Work out the finished part from the listing and answer in its coordinate system (mm). A direction names the side the tool comes from. Coordinates: 2 decimals unless noted, no trailing zeros. Order: outer loops, then holes, each group sorted by start corner. A loop starts at its lowest first (then second) coordinate and runs counter-clockwise, first axis right, second up. Notation, with made-up numbers: M 68,69 L 91,69 A18 ccw 91,83 Z; hole C 58.5,-31.75 d1. An arc over 180 degrees is marked long. Write item = value, one per line. Start each with the question number.
Q1. Each of these flat-tipped pins is pushed along its axis until it touches: P1, Ø8.5, axis at x = 59.32, y = 143.2, coming from the -Z side; P2, Ø10, axis at x = -100, z = 6.5, coming from the +Y side; P3, Ø16, axis at x = -155, y = 0, coming from the +Z side (3 decimals); P4, Ø8, axis at x = -121, z = 15.5, coming from the -Y side. Where does it stop, or does it pass through?
Q2. Determine the mould class of faces 1 (the cylindrical face through (149.547, 56.36, 24.145)), 2 (the flat face through (-2, -114, 0)) for opening direction X: released by +X, released by -X, zero draft, split by the parting line, or undercut.
Q3. Find section A-A on x = 0. Give the vertices of the cut face in (y, z) (3 decimals), and give its area (3 significant figures).
Q4. Find section C-C on z = 39.5. Give the number of separate pieces and of enclosed holes in the cut face, and give its area (3 significant figures).
Q5. Straight lines are drawn through the part: line 1 along Y through (x, z) = (0, 39); line 2 along X through (y, z) = (-57, 4); line 3 along Y through (x, z) = (147.5, 48.5). For each, find the intervals that lie inside material, in ascending order.
Q6. A tool of negligible diameter and unlimited length cuts with its end or side. For faces 3 (the flat face through (105, -9, 35)), 4 (the conical face through (92.016, 91.537, 4.202)), 5 (the flat face through (1, -100, 20)), from which of +Z, -Z, +X, -X, +Y, -Y can it reach the whole face along a straight path? Write none if from no direction.
```python
from build123d import *

# Parameters (mm, degrees)
SKETCH_1_R                    = 174
EXTRUDE_1_DEPTH               = 50
CUT_EXTRUDE_1_DEPTH           = 252.101573074
HOLE_WIZARD_M16_1_D           = 14
HOLE_WIZARD_M16_1_CSINK_D     = 16.05
HOLE_WIZARD_M16_1_CSINK_ANGLE = 90
PATTERN_CIRCULAR_1_COUNT      = 16
SKETCH_5_R                    = 130
CUT_EXTRUDE_2_DEPTH           = 15
CHAMFER_1_SIZE                = 2
CHAMFER_2_SIZE                = 5


with BuildPart() as part:
    # 草图1 → 凸台-拉伸1 (new body)
    with BuildSketch(Plane.XY):
        Circle(SKETCH_1_R)
    extrude(amount=EXTRUDE_1_DEPTH)

    # 草图2 → 切除-拉伸1 (cut, through all)
    with BuildSketch(Plane.XY.offset(50)):
        with BuildLine():
            Line((-70, 100), (70, 100))
            ThreePointArc((70, 100), (91.213203436, 91.213203436), (100, 70))
            Line((100, 70), (100, -70))
            ThreePointArc((100, -70), (91.213203436, -91.213203436), (70, -100))
            Line((70, -100), (-70, -100))
            ThreePointArc((-70, -100), (-91.213203436, -91.213203436), (-100, -70))
            Line((-100, -70), (-100, 70))
            ThreePointArc((-100, 70), (-91.213203436, 91.213203436), (-70, 100))
        make_face()
    extrude(amount=-CUT_EXTRUDE_1_DEPTH, mode=Mode.SUBTRACT)

    # M16 螺纹孔1 (through all)
    with Locations(Plane(origin=(0, 155, 50), x_dir=(1, 0, 0), z_dir=(0, 0, 1))):
        with Locations((0, 0)):
            hole_wizard_m16_1 = CounterSinkHole(HOLE_WIZARD_M16_1_D / 2, HOLE_WIZARD_M16_1_CSINK_D / 2, counter_sink_angle=HOLE_WIZARD_M16_1_CSINK_ANGLE)

    # 阵列(圆周)1: M16 螺纹孔1 ×16 about axis
    pattern_circular_1_axis = Axis((0, 0, 0), (0, 0, 1))
    for i in range(1, PATTERN_CIRCULAR_1_COUNT):
        add(hole_wizard_m16_1.rotate(pattern_circular_1_axis, i * 360 / PATTERN_CIRCULAR_1_COUNT), mode=Mode.SUBTRACT)

    # 草图5 → 切除-拉伸2 (cut)
    with BuildSketch(Plane.XY.offset(50)):
        Circle(SKETCH_5_R)
    extrude(amount=-CUT_EXTRUDE_2_DEPTH, mode=Mode.SUBTRACT)

    # 倒角1
    chamfer_1_edges = [part.edges().sort_by_distance(p)[0] for p in [
        (-130, 0, 50),
    ]]
    chamfer(chamfer_1_edges, length=CHAMFER_1_SIZE)

    # 倒角2
    chamfer_2_edges = [part.edges().sort_by_distance(p)[0] for p in [
        (-91.213203436, -91.213203436, 0),
        (-100, 0, 0),
        (-91.213203436, 91.213203436, 0),
        (0, 100, 0),
        (91.213203436, 91.213203436, 0),
        (100, 0, 0),
        (91.213203436, -91.213203436, 0),
        (0, -100, 0),
    ]]
    chamfer(chamfer_2_edges, length=CHAMFER_2_SIZE)


solid = part.part
```
Findings below:
q1.P1 = through
q1.P2 = 145.78
q1.P3 = 49.975
q1.P4 = -128.79
q2.face_1 = undercut
q2.face_2 = zero draft
q3.outline = M -174,0 L -162,0 L -162,48.975 L -163.025,50 L -174,50 Z; M -148,0 L -105,0 L -100,5 L -100,35 L -130,35 L -130,48 L -132,50 L -146.975,50 L -148,48.975 Z; M 100,5 L 105,0 L 148,0 L 148,48.975 L 146.975,50 L 132,50 L 130,48 L 130,35 L 100,35 Z; M 162,0 L 174,0 L 174,50 L 163.025,50 L 162,48.975 Z
q3.area = 5,070 mm^2
q4.separate_pieces = 1
q4.enclosed_holes = 17
q4.area = 39,600 mm^2
q5.line_1 = -174 to -162, -148 to -130, 130 to 148, 162 to 174
q5.line_2 = -164.4 to -149.81, -136.6 to -101, 101 to 136.6, 149.81 to 164.4
q5.line_3 = -92.3 to -64.84, -53.79 to 53.79, 64.84 to 92.3
q6.face_3 = +Z
q6.face_4 = -Z
q6.face_5 = +Z, -Z
